```python
from build123d import *

# Parameters (mm, degrees)
SKETCH_1_W                  = 135
SKETCH_1_H                  = 38
EXTRUDE_1_DEPTH             = 110
CUT_EXTRUDE_1_DEPTH         = 131.450182062
SKETCH_4_R                  = 11
CUT_EXTRUDE_2_DEPTH         = 4
SKETCH_5_R                  = 5.5
CUT_EXTRUDE_3_DEPTH         = 134.462541561
SKETCH_6_R                  = 7
CUT_EXTRUDE_4_DEPTH         = 4
PATTERN_LINEAR_1_COUNT      = 2
PATTERN_LINEAR_1_PITCH      = 60
PATTERN_LINEAR_1_COUNT_DIR2 = 2
PATTERN_LINEAR_1_PITCH_DIR2 = 72
PATTERN_LINEAR_2_COUNT      = 3
PATTERN_LINEAR_2_PITCH      = 27
PATTERN_LINEAR_2_COUNT_DIR2 = 2
PATTERN_LINEAR_2_PITCH_DIR2 = 76
CHAMFER_1_SIZE              = 4


with BuildPart() as part:
    # 草图1 → 凸台-拉伸1 (new body)
    with BuildSketch(Plane(origin=(0, 0, 0), x_dir=(1, 0, 0), z_dir=(0, 1, 0))):
        Rectangle(SKETCH_1_W, SKETCH_1_H)
    extrude(amount=EXTRUDE_1_DEPTH)

    # 草图3 → 切除-拉伸1 (cut, through all)
    with BuildSketch(Plane(origin=(0, 110, 0), x_dir=(1, 0, 0), z_dir=(0, 1, 0))):
        Polygon((20, 19), (-20, 19), (-20, 12), (-57.5, 12), (-57.5, -4), (-17, -4), (-17, -9), (17, -9), (17, -4), (57.5, -4), (57.5, 12), (20, 12), align=None)
    extrude(amount=-CUT_EXTRUDE_1_DEPTH, mode=Mode.SUBTRACT)

    # 草图4 → 切除-拉伸2 (cut)
    with BuildSketch(Plane(origin=(0, 0, -19), x_dir=(-1, 0, 0), z_dir=(0, 0, -1))):
        with Locations((-36, 85)):
            Circle(SKETCH_4_R)
    cut_extrude_2 = extrude(amount=-CUT_EXTRUDE_2_DEPTH, mode=Mode.SUBTRACT)

    # 草图5 → 切除-拉伸3 (cut, through all)
    with BuildSketch(Plane(origin=(0, 0, -15), x_dir=(-1, 0, 0), z_dir=(0, 0, -1))):
        with Locations((-36, 85)):
            Circle(SKETCH_5_R)
    cut_extrude_3 = extrude(amount=-CUT_EXTRUDE_3_DEPTH, mode=Mode.SUBTRACT)

    # 草图6 → 切除-拉伸4 (cut)
    with BuildSketch(Plane.XY.offset(19)):
        with Locations((36, 85)):
            Circle(SKETCH_6_R)
    cut_extrude_4 = extrude(amount=-CUT_EXTRUDE_4_DEPTH, mode=Mode.SUBTRACT)

    # 阵列(线性)1: 切除-拉伸2, 切除-拉伸3, Cut-Extrude 4 2 × 2
    with Locations(*[(-j * PATTERN_LINEAR_1_PITCH_DIR2, -i * PATTERN_LINEAR_1_PITCH, 0) for i in range(PATTERN_LINEAR_1_COUNT) for j in range(PATTERN_LINEAR_1_COUNT_DIR2) if (i, j) != (0, 0)]):
        add(cut_extrude_2, mode=Mode.SUBTRACT)
        add(cut_extrude_3, mode=Mode.SUBTRACT)
        add(cut_extrude_4, mode=Mode.SUBTRACT)

    # 草图7 → M6 螺纹孔1 (revolve, cut)
    with BuildSketch(Plane(origin=(27, 93, 19), x_dir=(0, -1, 0), z_dir=(1, 0, 0))):
        Polygon((0, 0), (0, 13.443375673), (2.5, 12), (2.5, 0), align=None)
    hole_wizard_m6_1 = revolve(axis=Axis((27, 93, 25.35), (0, 0, -1)), mode=Mode.SUBTRACT)

    # 阵列(线性)2: Hole Wizard M6 _1 3 × 2
    with Locations(*[(-i * PATTERN_LINEAR_2_PITCH, -j * PATTERN_LINEAR_2_PITCH_DIR2, 0) for i in range(PATTERN_LINEAR_2_COUNT) for j in range(PATTERN_LINEAR_2_COUNT_DIR2) if (i, j) != (0, 0)]):
        add(hole_wizard_m6_1, mode=Mode.SUBTRACT)

    # 倒角1
    chamfer_1_edges = [part.edges().sort_by_distance(p)[0] for p in [
        (-20, 55, -19),
        (20, 55, -19),
    ]]
    chamfer(chamfer_1_edges, length=CHAMFER_1_SIZE)


solid = part.part
```
Design review of the part built by this model. Coordinates are the model's own, in mm. A direction names the side the tool comes from. Coordinates: 2 decimals unless noted, no trailing zeros. Order: outer loops, then holes, each group sorted by start corner. A loop starts at its lowest first (then second) coordinate and runs counter-clockwise, first axis right, second up. Notation, with made-up numbers: M -5,-33.5 L 35,-33.5 A11 cw 35,-21.5 Z; hole C 52.5,18.5 d11. An arc over 180 degrees is marked long. Answer as a JSON object with one key per item and string values. Group by question number.
1) Add section D-D, the plane x = -36. Count the separate pieces of the cut face and the enclosed holes in it, then the cut area to 3 significant figures.
2) Wall thickness on L1, parallel to Y at x = -36, z = -14.2; L2, parallel to X at y = 89, z = -9.5; L3, parallel to X at y = 17, z = 13.5: over which ranges is each line inside the solid? List them lowest first.
3) For pin 1 (7 mm diameter, centred on x = -36.5, y = 82, fed in from +Z); pin 2 (6.5 mm diameter, centred on x = -37.5, y = 82.5, fed in from -Z), all flat-tipped, find the tip position at first contact; note any pin that passes through.
4) Add section B-B, the plane z = 0. Write out the cut boundary in (x, y), then the cut area to 3 significant figures.
5) Add section A-A, the plane x = 22. Write out the cut boundary in (y, z), then the cut area to 3 significant figures.
6) Add section C-C, the plane y = 12.5. Write out the cut boundary in (x, z).
7) Mouldability with a two-part tool opening along Y and no side actions: class faces 6 (the cylindrical face through (-36.91, 91.94, 17.03)), 7 (the conical face through (-27.13, 92.586, 5.807)), 8 (the flat face through (-1, 110, 12)), 9 (the flat face through (17, 56, 7)) as pulls with the +Y half, pulls with the -Y half, needs draft (parallel to the pull), parting line crosses it, or undercut.
8) Tool access review of faces 1 (the cylindrical face through (-35.284, 90.453, 9.423)), 2 (the flat face through (41, 88, -15)), 3 (the flat face through (-38, 56, 4)), 4 (the cylindrical face through (-27.1, 95.5, 13.1)), 5 (the flat face through (-20, 56, -14)): name each direction out of +Z, -Z, +X, -X, +Y, -Y from which nothing blocks a thin tool from reaching the whole face with its end or side.
Computed values:
{
 "1": {"separate pieces": "6", "enclosed holes": "0", "area": "1,820 mm^2"},
 "2": {"L1": "y = 0 to 19.5, 30.5 to 79.5, 90.5 to 110", "L2": "x = -67.5 to -57.5, 57.5 to 67.5", "L3": "x = -67.5 to -29.5, -24.5 to -2.5, 2.5 to 24.5, 29.5 to 67.5"},
 "3": {"pin 1": "stops at z = 15", "pin 2": "stops at z = -15"},
 "4": {"outline": "M -67.5,0 L -57.5,0 L -57.5,110 L -67.5,110 Z; M 57.5,0 L 67.5,0 L 67.5,110 L 57.5,110 Z", "area": "2,200 mm^2"},
 "5": {"outline": "M 0,-17 L 110,-17 L 110,-12 L 0,-12 Z; M 0,4 L 110,4 L 110,19 L 0,19 Z", "area": "2,200 mm^2"},
 "6": {"outline": "M -67.5,-19 L -24,-19 L -20,-15 L -20,-12 L -57.5,-12 L -57.5,4 L -17,4 L -17,9 L 17,9 L 17,4 L 57.5,4 L 57.5,-12 L 20,-12 L 20,-15 L 24,-19 L 67.5,-19 L 67.5,19 L -67.5,19 Z"},
 "7": {"face 6": "undercut", "face 7": "undercut", "face 8": "pulls with the +Y half", "face 9": "needs draft"},
 "8": {"face 1": "+Z, -Z", "face 2": "-Z", "face 3": "+Y, -Y", "face 4": "+Z", "face 5": "-Z, +Y, -Y"}
}
